from build123d import *

# Parameters (mm, degrees)
SKETCH1_R           = 5
BOSS_EXTRUDE1_DEPTH = 30
SKETCH2_R           = 10
BOSS_EXTRUDE2_DEPTH = 12
CUT_EXTRUDE1_DEPTH  = 8


with BuildPart() as part:
    # Sketch1 → Boss-Extrude1 (new body)
    with BuildSketch(Plane(origin=(0, 0, 0), x_dir=(1, 0, 0), z_dir=(0, 1, 0))):
        with Locations(Location((0, 0, 0), (0, 0, 270))):
            Circle(SKETCH1_R)
    extrude(amount=BOSS_EXTRUDE1_DEPTH)

    # Sketch2 → Boss-Extrude2 (add)
    with BuildSketch(Plane(origin=(0, 30, 0), x_dir=(1, 0, 0), z_dir=(0, 1, 0))):
        with Locations(Location((0, 0, 0), (0, 0, 270))):
            Circle(SKETCH2_R)
    extrude(amount=BOSS_EXTRUDE2_DEPTH)

    # Sketch3 → Cut-Extrude1 (cut)
    with BuildSketch(Plane(origin=(0, 42, 0), x_dir=(1, 0, 0), z_dir=(0, 1, 0))):
        Polygon((4.59389972, -4.318555573), (6.036928694, 1.819156074), (1.443028974, 6.137711647), (-4.59389972, 4.318555573), (-6.036928694, -1.819156074), (-1.443028974, -6.137711647), align=None)
    extrude(amount=-CUT_EXTRUDE1_DEPTH, mode=Mode.SUBTRACT)


solid = part.part
Input: part model. Units: mm. Frame: model coordinates. A direction names the side the tool comes from. Give positions to 0.01 mm unless a question says otherwise; leave off trailing zeros. Loops run counter-clockwise (first coordinate to the right, second up) from the corner with the lowest first, then second, coordinate; pieces in that order, holes last. Notation, with made-up numbers: (-13, -13.5) - (-8, -13.5) arc R22 ccw to (-8, 5.5) - close; hole circle Ø5 at (24.5, -7). An arc over 180 degrees is marked (long way). Use CSV: the item, a comma, the result in double quotes. Start each with the question number.
Item 1: Section C-C on z = 0. Return loops of the section in (x, y), then the cut area to 3 significant figures.
Item 2: Contact query for flat-ended pins moving along their axis: P1, Ø3, axis at y = 20.5, z = 0.5, coming from the +X side; P2, Ø12, axis at x = -2.5, z = 0.5, coming from the +Y side; P3, Ø5, axis at x = 3.5, y = 29.5, coming from the -Z side; P4, Ø8, axis at x = 6.5, y = 32.5, coming from the -Z side. Output: stop coordinate, or through.
Item 3: Mould query, pull axis X, two halves, no side actions, for faces 4 (the flat face through (5.305, 38.056, 1.293)), 5 (the cylindrical face through (-4.88, 14.79, -1.08)), 6 (the flat face through (0, 0, 0)). Classes: pulls with the +X half, pulls with the -X half, needs draft (parallel to the pull), parting line crosses it, or undercut.
Item 4: Section B-B on x = -2.5. Return loops of the section in (y, z), then the cut area to 3 significant figures.
Item 5: Section A-A on y = 36. Return loops of the section in (x, z).
Item 6: Section D-D on y = 31.5. Return loops of the section in (x, z), then the cut area to 3 significant figures.
Item 7: Line query: line 1 (Y direction, x = 2.25, z = 1); line 2 (Y direction, x = 1.5, z = 5); line 3 (X direction, y = 19.5, z = 4.25). Output: solid intervals per line, ascending.
Item 8: Reachability of faces 1 (the flat face through (5, 30, 2)), 2 (the cylindrical face through (-9.76, 35.92, -2.17)), 3 (the flat face through (0, 34, 0)) from +Z, -Z, +X, -X, +Y, -Y: full face, straight path, thin tool, end or side. Return the list, or none.
Ans:
1,outline,"(-10, 30) - (-5, 30) - (-5, 0) - (5, 0) - (5, 30) - (10, 30) - (10, 42) - (5.61, 42) - (5.61, 34) - (-5.61, 34) - (-5.61, 42) - (-10, 42) - close"
1,area,"450 mm2"
2,P1,"stops at x = 5"
2,P2,"stops at y = 42"
2,P3,"stops at z = -9.94"
2,P4,"stops at z = -9.68"
3,face 4,"undercut"
3,face 5,"parting line crosses it"
3,face 6,"needs draft"
4,outline,"(0, -4.33) - (30, -4.33) - (30, -9.68) - (42, -9.68) - (42, -4.95) - (34, -4.95) - (34, 5.14) - (42, 5.14) - (42, 9.68) - (30, 9.68) - (30, 4.33) - (0, 4.33) - close"
4,area,"411 mm2"
5,outline,"circle Ø20 at (0, 0); hole (-6.04, 1.82) - (-4.59, -4.32) - (1.44, -6.14) - (6.04, -1.82) - (4.59, 4.32) - (-1.44, 6.14) - close"
6,outline,"circle Ø20 at (0, 0)"
6,area,"314 mm2"
7,line 1,"y = 0 to 34"
7,line 2,"y = 30 to 34"
7,line 3,"x = -2.63 to 2.63"
8,face 1,"-Y"
8,face 2,"+Y, -Y"
8,face 3,"+Y"
